Here's how the part is built. I have some questions about the finished solid (model axes, mm). Face numbers are marked on the shaded views. Give positions to 0.01 mm unless a question says otherwise; leave off trailing zeros. Write each loop counter-clockwise with the first axis right and the second up, starting at its lowest first coordinate (ties: lowest second). Pieces come first, ordered by that corner, then holes. Notation, with made-up numbers: (-36.5, 28) -> (-22.5, 28) arc R14 ccw to (-22.5, 38) -> close; hole circle Ø4 at (40.25, -27). An arc over 180 degrees is marked (long way). Use one line per item in the form item = value.
```python
from build123d import *

# Parameters (mm, degrees)
BOSS_EXTRUDE1_DEPTH     = 200
CUT_EXTRUDE1_DEPTH      = 254.860197747
CUT_EXTRUDE1_DEPTH_BACK = 254.860197747
SKETCH3_R               = 2.5
FILLET1_R               = 5
CUT_EXTRUDE2_DEPTH      = 254.860197747
CUT_EXTRUDE2_DEPTH_BACK = 254.860197747
SKETCH5_R               = 2.5


with BuildPart() as part:
    # Sketch2 → Boss-Extrude1 (new body)
    with BuildSketch(Plane(origin=(0, 50, 0), x_dir=(1, 0, 0), z_dir=(0, 1, 0))):
        Polygon((35, 10), (35, 20), (27, 20), (27, 22), (37, 22), (37, -2), (27, -2), (27, 0), (35, 0), align=None)
    extrude(amount=BOSS_EXTRUDE1_DEPTH)

    # Sketch3 → Cut-Extrude1 (cut, two sides: drawn at the far end of the back side and taken through both)
    with BuildSketch(Plane.XY.offset(2).offset(-CUT_EXTRUDE1_DEPTH_BACK)):
        with Locations((30, 55)):
            Circle(SKETCH3_R)
    extrude(amount=CUT_EXTRUDE1_DEPTH + CUT_EXTRUDE1_DEPTH_BACK, mode=Mode.SUBTRACT)

    # Fillet1
    fillet1_edges = [part.edges().sort_by_distance(p)[0] for p in [
        (27, 250, 1),
        (27, 250, -21),
    ]]
    fillet(fillet1_edges, radius=FILLET1_R)

    # Sketch5 → Cut-Extrude2 (cut, two sides: drawn at the far end of the back side and taken through both)
    with BuildSketch(Plane.XY.offset(2).offset(-CUT_EXTRUDE2_DEPTH_BACK)):
        with Locations((32, 245)):
            Circle(SKETCH5_R)
    extrude(amount=CUT_EXTRUDE2_DEPTH + CUT_EXTRUDE2_DEPTH_BACK, mode=Mode.SUBTRACT)


solid = part.part
```
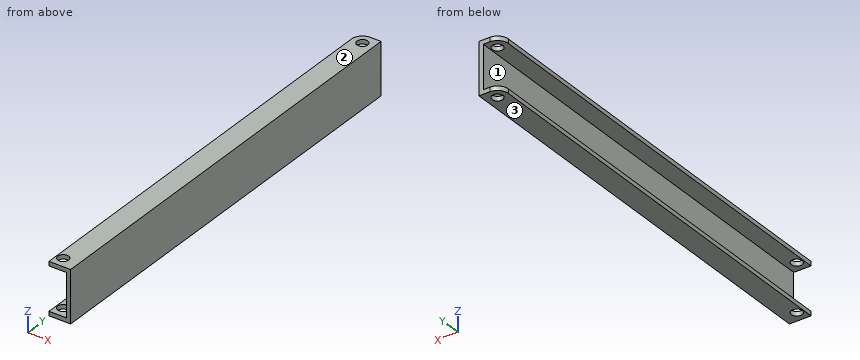
Q1. If I drill on line 1 along Z through (x, y) = (31.5, 103); line 2 along Y through (x, z) = (30, -21.6); line 3 along X through (y, z) = (245, -21.35), over which ranges is the centre line in solid material (lowest first)? Write a range as from..to.
Result set:
line_1 = -22..-20, 0..2
line_2 = 50..52.5, 57.5..243.5, 246.5..249.58
line_3 = 27..29.5, 34.5..37
Q2. I want a section at A-A, the plane y = 160. Write out the boundary of the cut face in (x, z), and give its area (3 significant figures).
Result set:
outline = (27, -22) -> (37, -22) -> (37, 2) -> (27, 2) -> (27, 0) -> (35, 0) -> (35, -20) -> (27, -20) -> close
area = 80.0 mm2
Q3. If we mould it in two halves opening along Z, with no side actions, what happens to the marked faces 1, 2 and 3? For each: +Z half, -Z half, draft (parallel to the pull), parting line (faces both ways), or undercut.
Result set:
face_1 = undercut
face_2 = +Z half
face_3 = -Z half
Q4. I want a section at B-B, the plane z = -11.75. Write out the boundary of the cut face in (x, y).
Result set:
outline = (35, 50) -> (37, 50) -> (37, 250) -> (35, 250) -> close
Q5. Will this pin go through, and if not, where does the flat tip stop? pin 1 Ø4 at (y, z) = (120, -16) entering from -X.
Result set:
pin_1 = 35
